from build123d import *

# Parameters (mm, degrees)
SKETCH_1_W          = 100
SKETCH_1_H          = 140
EXTRUDE_1_DEPTH     = 14
CUT_EXTRUDE_1_REACH = 89.155
SKETCH_2_R          = 39
SKETCH_3_W          = 8
SKETCH_3_H          = 140
EXTRUDE_2_DEPTH     = 12


with BuildPart() as part:
    # 草图1 → 凸台-拉伸1 (new body)
    with BuildSketch(Plane.XY):
        Rectangle(SKETCH_1_W, SKETCH_1_H)
    extrude(amount=EXTRUDE_1_DEPTH)

    # 草图2 → 切除-拉伸1 (cut, up to next)
    with BuildSketch(Plane.XY.offset(14), mode=Mode.PRIVATE) as cut_extrude_1_sk1:
        with Locations((4, 24)):
            Circle(SKETCH_2_R)
    cut_extrude_1_tool1 = extrude(cut_extrude_1_sk1.sketch, amount=-CUT_EXTRUDE_1_REACH, mode=Mode.PRIVATE) & part.part
    add(cut_extrude_1_tool1.solids().sort_by_distance((4, 24, 14))[0], mode=Mode.SUBTRACT)

    # 草图3 → 凸台-拉伸2 (add)
    with BuildSketch(Plane.XY.offset(14)):
        with Locations((-46, 0)):
            Rectangle(SKETCH_3_W, SKETCH_3_H)
    extrude(amount=EXTRUDE_2_DEPTH)


solid = part.part
Here's how the part is built. I have some questions about the finished solid (model axes, mm). A direction names the side the tool comes from. Coordinates: 2 decimals unless noted, no trailing zeros. Loops run counter-clockwise (first coordinate to the right, second up) from the corner with the lowest first, then second, coordinate; pieces in that order, holes last.
1. Imagine slicing it at A-A, the plane y = 24. Please give me the cut outline in (x, z), and give its area (3 significant figures).
2. If we mould it in two halves opening along Y, with no side actions, what happens to faces 1 (the flat face through (-1, -70, 7)), 2 (the flat face through (-1, 70, 7)), 3 (the cylindrical face through (-4.454, -14.073, 7.098)), 4 (the flat face through (-12, -15, 0))? For each: pulls with the +Y half, pulls with the -Y half, needs draft (parallel to the pull), parting line crosses it, or undercut.
3. For P1, Ø12, axis at x = -3, y = 51, coming from the +Z side; P2, Ø5, axis at x = 20, y = -53, coming from the -Z side, each with a flat end and sliding along its axis, tell me the tip position at first contact or that it passes through.
4. Imagine slicing it at D-D, the plane x = 40. Please give me the cut outline in (y, z).
5. Imagine slicing it at B-B, the plane x = 4. Please give me the cut outline in (y, z).
6. Imagine slicing it at C-C, the plane z = 11.75. Please give me the cut outline in (x, y), and give its area (3 significant figures).
7. I need wall thicknesses on L1, parallel to Z at x = 22.5, y = -64; L2, parallel to X at y = 24.5, z = 24; L3, parallel to Y at x = 4, z = 3. Which ranges of each line are inside material? Lowest first, please.
8. For faces 5 (the flat face through (-7, -15, 14)), 6 (the flat face through (50, -1, 7)), which set-ups out of +Z, -Z, +X, -X, +Y, -Y let a thin tool reach every point of the face, with its end or its side?
Taken from the geometry:
1. outline: (-50, 0) - (-35, 0) - (-35, 14) - (-42, 14) - (-42, 26) - (-50, 26) - close; (43, 0) - (50, 0) - (50, 14) - (43, 14) - close
1. area: 404 mm2
2. face 1: pulls with the -Y half
2. face 2: pulls with the +Y half
2. face 3: undercut
2. face 4: needs draft
3. P1: passes through
3. P2: stops at z = 0
4. outline: (-70, 0) - (9, 0) - (9, 14) - (-70, 14) - close; (39, 0) - (70, 0) - (70, 14) - (39, 14) - close
5. outline: (-70, 0) - (-15, 0) - (-15, 14) - (-70, 14) - close; (63, 0) - (70, 0) - (70, 14) - (63, 14) - close
6. outline: (-50, -70) - (50, -70) - (50, 70) - (-50, 70) - close; hole circle Ø78 at (4, 24)
6. area: 9,220 mm2
7. L1: z = 0 to 14
7. L2: x = -50 to -42
7. L3: y = -70 to -15, 63 to 70
8. face 5: +Z, +X, +Y, -Y
8. face 6: +Z, -Z, +X, +Y, -Y
